The listing builds one solid part. Answer for the finished solid, in the listing's coordinates (mm). A direction names the side the tool comes from. Give positions to 0.01 mm unless a question says otherwise; leave off trailing zeros. Write each loop counter-clockwise with the first axis right and the second up, starting at its lowest first coordinate (ties: lowest second). Pieces come first, ordered by that corner, then holes.
```python
from build123d import *

# Parameters (mm, degrees)
HUB_BOSSES_20MM_DEPTH        = 10
HUB_BOSSES_20MM_DEPTH_BACK   = 10
HUB_BOSSES_20MM_2_DEPTH      = 10
HUB_BOSSES_20MM_2_DEPTH_BACK = 10
LEVER_PROFILE_SKETCH_R       = 10
ARM_WEB_10MM_DEPTH           = 5
ARM_WEB_10MM_DEPTH_BACK      = 5


with BuildPart() as part:
    # Lever Profile Sketch → Hub Bosses 20mm (new, two sides: drawn at the far end of the back side and taken through both)
    with BuildSketch(Plane.XY.offset(-HUB_BOSSES_20MM_DEPTH_BACK)):
        with BuildLine():
            ThreePointArc((-123.274285714, 23.791815434), (-128.116796704, -19.121027957), (-85.057142857, -22.411658773))
            ThreePointArc((-85.057142857, -22.411658773), (-77.629525814, -12.282391577), (-75, 0))
            ThreePointArc((-75, 0), (-75.077467799, 2.154545592), (-75.309471114, 4.297963991))
            ThreePointArc((-75.309471114, 4.297963991), (-78.312822706, 13.703815821), (-84.206993671, 21.625237289))
            ThreePointArc((-84.206993671, 21.625237289), (-103.338824634, 29.953972965), (-123.274285714, 23.791815434))
        make_face()
        with BuildLine():
            Line((-109, 14.456832295), (-109, 20.578458237))
            Line((-109, 20.578458237), (-101, 20.578458237))
            Line((-101, 20.578458237), (-101, 14.456832295))
            ThreePointArc((-101, 14.456832295), (-105, -15), (-109, 14.456832295))
        make_face(mode=Mode.SUBTRACT)
    extrude(amount=HUB_BOSSES_20MM_DEPTH + HUB_BOSSES_20MM_DEPTH_BACK)



with BuildPart() as body_2:
    # Lever Profile Sketch → Hub Bosses 20mm 2 (new, two sides: drawn at the far end of the back side and taken through both)
    with BuildSketch(Plane.XY.offset(-HUB_BOSSES_20MM_2_DEPTH_BACK)):
        with BuildLine():
            ThreePointArc((-20.407235595, 4.954264362), (-19.57486428, -7.604254627), (-11.711111111, -17.431290157))
            ThreePointArc((-11.711111111, -17.431290157), (9.875896584, -18.532853711), (21, 0))
            ThreePointArc((21, 0), (19.39587585, 8.049844719), (14.828571429, 14.869884646))
            ThreePointArc((14.828571429, 14.869884646), (0.022511477, 20.999987934), (-14.796657075, 14.901642172))
            ThreePointArc((-14.796657075, 14.901642172), (-18.291148026, 10.316680857), (-20.407235595, 4.954264362))
        make_face()
        Circle(LEVER_PROFILE_SKETCH_R, mode=Mode.SUBTRACT)
    extrude(amount=HUB_BOSSES_20MM_2_DEPTH + HUB_BOSSES_20MM_2_DEPTH_BACK)


with BuildPart() as part_1:
    add(part.part)

    add(body_2.part)  # Arm Web 10mm merges body 2
    # Sketch1_6 → Arm Web 10mm (add, two sides: drawn at the far end of the back side and taken through both)
    with BuildSketch(Plane.XY.offset(-ARM_WEB_10MM_DEPTH_BACK)):
        with BuildLine():
            ThreePointArc((-85.057142857, -22.411658773), (-49.236210113, -7.37282174), (-11.711111111, -17.431290157))
            ThreePointArc((-11.711111111, -17.431290157), (-19.57486428, -7.604254627), (-20.407235595, 4.954264362))
            ThreePointArc((-20.407235595, 4.954264362), (-23.975479097, 0.036453925), (-29.969842477, -0.955931516))
            ThreePointArc((-29.969842477, -0.955931516), (-47.593498278, 0.721874536), (-65.052989568, -2.206340072))
            ThreePointArc((-65.052989568, -2.206340072), (-71.676423998, -1.311923165), (-75.309471114, 4.297963991))
            ThreePointArc((-75.309471114, 4.297963991), (-75.077467799, 2.154545592), (-75, 0))
            ThreePointArc((-75, 0), (-77.629525814, -12.282391577), (-85.057142857, -22.411658773))
        make_face()
        with BuildLine():
            ThreePointArc((-14.796657075, 14.901642172), (0.022511477, 20.999987934), (14.828571429, 14.869884646))
            ThreePointArc((14.828571429, 14.869884646), (-52.545027473, 45.302030133), (-123.274285714, 23.791815434))
            ThreePointArc((-123.274285714, 23.791815434), (-103.338824634, 29.953972965), (-84.206993671, 21.625237289))
            ThreePointArc((-84.206993671, 21.625237289), (-86.365233313, 29.551401021), (-80.401329626, 35.200641913))
            ThreePointArc((-80.401329626, 35.200641913), (-48.040951998, 36.863141194), (-16.938574827, 27.77468267))
            ThreePointArc((-16.938574827, 27.77468267), (-12.541970936, 21.891509402), (-14.796657075, 14.901642172))
        make_face()
    extrude(amount=ARM_WEB_10MM_DEPTH + ARM_WEB_10MM_DEPTH_BACK)


solid = part_1.part
```
Item 1: A cutting plane is placed at A-A, the plane z = 7.5. Give the vertices of the cut face in (x, y), plus the area to 3 significant figures.
Conclusion:
outline: circle Ø60 at (-105, 0); circle Ø42 at (0, 0); hole (-109, 14.46) arc R15 ccw (long way) to (-101, 14.46) - (-101, 20.58) - (-109, 20.58) - close; hole circle Ø20 at (0, 0)
area: 3,150 mm2
Item 2: Each of these flat-tipped pins is pushed along its axis until it touches: P1, Ø24.5, axis at x = -33.5, y = 28, coming from the -Z side; P2, Ø10, axis at y = 25, z = -7.5, coming from the -X side; P3, Ø6.5, axis at y = 18.5, z = 2, coming from the -X side. Where does it stop, or does it pass through?
Conclusion:
P1: stops at z = -5
P2: stops at x = -127.36
P3: stops at x = -130.83
Item 3: A cutting plane is placed at B-B, the plane x = -82. Give the vertices of the cut face in (y, z).
Conclusion:
outline: (-19.87, -5) - (-19.26, -5) - (-19.26, -10) - (19.26, -10) - (19.26, 10) - (-19.26, 10) - (-19.26, 5) - (-19.87, 5) - close; (34.66, -5) - (43.04, -5) - (43.04, 5) - (34.66, 5) - close
Item 4: Determine the mould class of faces 3 (the face through (-51.49, 45.23, -0.07)), 4 (the face through (-109, 17, 0)), 5 (the face through (-5, -9, -10)) for opening direction X: pulls with the +X half, pulls with the -X half, needs draft (parallel to the pull), parting line crosses it, or undercut.
Conclusion:
face 3: parting line crosses it
face 4: undercut
face 5: needs draft
Item 5: A cutting plane is placed at C-C, the plane x = -24.5. Give the vertices of the cut face in (y, z).
Conclusion:
outline: (-10.91, -5) - (-0.26, -5) - (-0.26, 5) - (-10.91, 5) - close; (31.06, -5) - (39.58, -5) - (39.58, 5) - (31.06, 5) - close
Item 6: Consider probe 1 along X at (y, z) = (20, -1.5); probe 2 along X at (y, z) = (-12, -6); probe 3 along X at (y, z) = (5, -3). Determine where each line is inside the solid, lowest interval first.
Conclusion:
probe 1: x = -127.36 to -109, -101 to -82.64, -12.45 to 9.3
probe 2: x = -132.5 to -114, -96 to -77.5, -17.23 to 17.23
probe 3: x = -134.58 to -119.14, -90.86 to -75.42, -20.4 to -8.66, 8.66 to 20.4
Item 7: A cutting plane is placed at D-D, the plane x = -105. Give the vertices of the cut face in (y, z).
Conclusion:
outline: (-30, -10) - (-15, -10) - (-15, 10) - (-30, 10) - close; (20.58, -10) - (30, -10) - (30, -5) - (35.06, -5) - (35.06, 5) - (30, 5) - (30, 10) - (20.58, 10) - close
Item 8: Which of the six approach directions +Z, -Z, +X, -X, +Y, -Y give full straight-line access (tool end or side, diameter ignored) to faces 1 (the face through (-5, -9, 10)), 2 (the face through (-23.902, 0.083, -0.07))?
Conclusion:
face 1: +Z, +X, -X, +Y, -Y
face 2: +Z, -Z
